from build123d import *

# Parameters (mm, degrees)
BASE_PLATE_SKETCH_W    = 110
BASE_PLATE_SKETCH_H    = 55
BASE_PLATE_SKETCH_R    = 5
BASE_PLATE_DEPTH       = 15
V_BLOCK_UPRIGHTS_DEPTH = 55
UPRIGHT_NOTCH_SKETCH_W = 12
UPRIGHT_NOTCH_SKETCH_H = 5
UPRIGHT_NOTCH_DEPTH    = 108.791465339
ANGLED_CUT_30DEG_DEPTH = 12


with BuildPart() as part:
    # Base Plate Sketch → Base Plate (new body)
    with BuildSketch(Plane(origin=(0, 0, 0), x_dir=(1, 0, 0), z_dir=(0, 1, 0))):
        with Locations((0, 27.5)):
            Rectangle(BASE_PLATE_SKETCH_W, BASE_PLATE_SKETCH_H)
        with Locations(Location((-42, 40, 0), (0, 0, 270))):
            Circle(BASE_PLATE_SKETCH_R, mode=Mode.SUBTRACT)
        with Locations(Location((-42, 20, 0), (0, 0, 270))):
            Circle(BASE_PLATE_SKETCH_R, mode=Mode.SUBTRACT)
        with Locations(Location((42, 20, 0), (0, 0, 90))):
            Circle(BASE_PLATE_SKETCH_R, mode=Mode.SUBTRACT)
        with Locations(Location((42, 40, 0), (0, 0, 90))):
            Circle(BASE_PLATE_SKETCH_R, mode=Mode.SUBTRACT)
    extrude(amount=BASE_PLATE_DEPTH)

    # V-Block Uprights Sketch → V-Block Uprights (add)
    with BuildSketch(Plane(origin=(0, 0, -55), x_dir=(-1, 0, 0), z_dir=(0, 0, -1))):
        Polygon((-30, 15), (-18, 15), (18, 15), (30, 15), (30, 37), (18, 37), (18, 19.5), (-18, 19.5), (-18, 37), (-30, 37), align=None)
    extrude(amount=-V_BLOCK_UPRIGHTS_DEPTH)

    # Upright Notch Sketch → Upright Notch (cut, through all)
    with BuildSketch(Plane.ZY.offset(30)):
        Polygon((0, 15), (-28, 37), (0, 37), align=None)
        with Locations((-49, 34.5)):
            Rectangle(UPRIGHT_NOTCH_SKETCH_W, UPRIGHT_NOTCH_SKETCH_H)
    extrude(amount=-UPRIGHT_NOTCH_DEPTH, mode=Mode.SUBTRACT)

    # Angled Cut 30deg Sketch → Angled Cut 30deg (cut)
    with BuildSketch(Plane.ZY.offset(-18)):
        Polygon((-55, 19.5), (-47.783121635, 32), (-55, 32), align=None)
    extrude(amount=-ANGLED_CUT_30DEG_DEPTH, mode=Mode.SUBTRACT)


solid = part.part
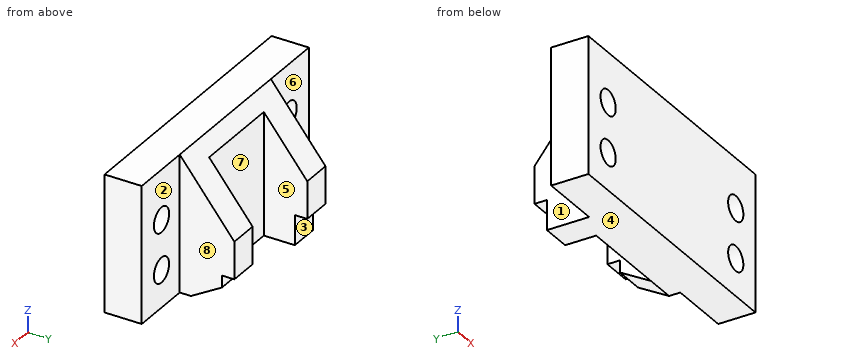
Design review of the part built by this model. Coordinates are the model's own, in mm. Face numbers are marked on the shaded views. A direction names the side the tool comes from. Round coordinates to 2 decimals unless told otherwise and drop trailing zeros. Write each loop counter-clockwise with the first axis right and the second up, starting at its lowest first coordinate (ties: lowest second). Pieces come first, ordered by that corner, then holes.
Item 1: Consider section A-A on x = 42. Give the boundary of the cut face in (y, z), and give its area (3 significant figures).
Item 2: For pin 1 Ø13 at (x, z) = (-23.5, -51) entering from +Y; pin 2 Ø19 at (y, z) = (30, -20.5) entering from -X; pin 3 Ø17.5 at (y, z) = (29, -23) entering from +X; pin 4 Ø4 at (x, y) = (10.5, 6.5) entering from +Z, all flat-tipped, find the tip position at first contact; note any pin that passes through.
Item 3: Draft analysis for pull direction X (two halves, no side actions). For the marked faces 5, 6, 7 and 8, state which applies: released by +X, released by -X, zero draft, split by the parting line, or undercut.
Item 4: For the marked faces 1, 2, 3 and 4, list the 3-axis set-ups (+Z, -Z, +X, -X, +Y, -Y) from which the entire face can be reached by the end or side of a thin tool; tool diameter is ignored.
Item 5: Wall thickness on L1, parallel to Z at x = 42, y = 7.75; L2, parallel to X at y = 7, z = -20; L3, parallel to X at y = 23, z = -42: over which ranges is each line inside the solid? List them lowest first.
Item 6: Consider section D-D on z = -32. Give the boundary of the cut face in (x, y), and give its area (3 significant figures).
Item 7: Consider section C-C on y = 30. Give the boundary of the cut face in (x, z), and give its area (3 significant figures).
Item 8: Consider section B-B on z = -40. Give the boundary of the cut face in (x, y).
Check values:
1. outline: (0, -55) - (15, -55) - (15, -45) - (0, -45) - close; (0, -35) - (15, -35) - (15, -25) - (0, -25) - close; (0, -15) - (15, -15) - (15, 0) - (0, 0) - close
1. area: 525 mm2
2. pin 1: stops at y = 32
2. pin 2: stops at x = -30
2. pin 3: stops at x = 30
2. pin 4: stops at z = 0
3. face 5: undercut
3. face 6: zero draft
3. face 7: undercut
3. face 8: released by +X
4. face 1: +Z, -Z, -X, +Y
4. face 2: +Z, -Z, +X, +Y
4. face 3: -Z, +X, -X, +Y
4. face 4: -Z, +X, -X, +Y, -Y
5. L1: z = -55 to -45, -35 to -25, -15 to 0
5. L2: x = -55 to -47, -37 to 37, 47 to 55
5. L3: x = -30 to -18, 18 to 30
6. outline: (-55, 0) - (55, 0) - (55, 15) - (30, 15) - (30, 37) - (18, 37) - (18, 19.5) - (-18, 19.5) - (-18, 37) - (-30, 37) - (-30, 15) - (-55, 15) - close
6. area: 2,340 mm2
7. outline: (-30, -55) - (-18, -55) - (-18, -19.09) - (-30, -19.09) - close; (18, -48.94) - (30, -48.94) - (30, -19.09) - (18, -19.09) - close
7. area: 789 mm2
8. outline: (-55, 0) - (-47, 0) - (-47, 15) - (-55, 15) - close; (-37, 0) - (37, 0) - (37, 15) - (30, 15) - (30, 37) - (18, 37) - (18, 19.5) - (-18, 19.5) - (-18, 37) - (-30, 37) - (-30, 15) - (-37, 15) - close; (47, 0) - (55, 0) - (55, 15) - (47, 15) - close
